Check sheet for the modelled part. Datum: model origin and axes. Units: mm. Coordinates: 2 decimals unless noted, no trailing zeros. Order: outer loops, then holes, each group sorted by start corner. A loop starts at its lowest first (then second) coordinate and runs counter-clockwise, first axis right, second up.
1. Thickness scan on line 1 (Y direction, x = -106.4, z = 2.25). Record the ranges inside material, lowest first.
2. Cross-section at B-B (x = -106.4). Enter the section's corners in (y, z), then the cut area to 3 significant figures.
3. Cross-section at A-A (y = 52.35). Enter the section's corners in (x, z), then the cut area to 3 significant figures.
4. Draft check along Y on faces 1 (the flat face through (-2, 1, 0)), 2 (the flat face through (-2, -72, 3)), 3 (the cylindrical face through (109.357, -47.712, 3.042)). Enter one of: released by +Y, released by -Y, zero draft, split by the parting line, or undercut.
```python
from build123d import *

# Parameters (mm, degrees)
SKETCH1_W            = 240
SKETCH1_H            = 144
BOSS_EXTRUDE1_DEPTH  = 6
SKETCH2_R            = 5.5
CUT_EXTRUDE1_DEPTH   = 6
LPATTERN1_COUNT      = 2
LPATTERN1_PITCH      = 212.8
LPATTERN1_COUNT_DIR2 = 2
LPATTERN1_PITCH_DIR2 = 104.7


with BuildPart() as part:
    # Sketch1 → Boss-Extrude1 (new body)
    with BuildSketch(Plane.XY):
        Rectangle(SKETCH1_W, SKETCH1_H)
    extrude(amount=BOSS_EXTRUDE1_DEPTH)

    # Sketch2 → Cut-Extrude1 (cut)
    with BuildSketch(Plane.XY.offset(6)):
        with Locations((-106.4, 52.35)):
            Circle(SKETCH2_R)
    cut_extrude1 = extrude(amount=-CUT_EXTRUDE1_DEPTH, mode=Mode.SUBTRACT)

    # LPattern1: Cut-Extrude1 2 × 2
    with Locations(*[(i * LPATTERN1_PITCH, -j * LPATTERN1_PITCH_DIR2, 0) for i in range(LPATTERN1_COUNT) for j in range(LPATTERN1_COUNT_DIR2) if (i, j) != (0, 0)]):
        add(cut_extrude1, mode=Mode.SUBTRACT)


solid = part.part
```
Data:
1. line 1: y = -72 to -57.85, -46.85 to 46.85, 57.85 to 72
2. outline: (-72, 0) - (-57.85, 0) - (-57.85, 6) - (-72, 6) - close; (-46.85, 0) - (46.85, 0) - (46.85, 6) - (-46.85, 6) - close; (57.85, 0) - (72, 0) - (72, 6) - (57.85, 6) - close
2. area: 732 mm2
3. outline: (-120, 0) - (-111.9, 0) - (-111.9, 6) - (-120, 6) - close; (-100.9, 0) - (100.9, 0) - (100.9, 6) - (-100.9, 6) - close; (111.9, 0) - (120, 0) - (120, 6) - (111.9, 6) - close
3. area: 1,310 mm2
4. face 1: zero draft
4. face 2: released by -Y
4. face 3: undercut
